Can you work these out from the model? Positions are in its coordinate system, mm. Round coordinates to 2 decimals unless told otherwise and drop trailing zeros. Loops run counter-clockwise (first coordinate to the right, second up) from the corner with the lowest first, then second, coordinate; pieces in that order, holes last. Notation, with made-up numbers: M -29,-1.75 L 4,-1.75 A28 ccw 4,28.25 Z; hole C 19.25,46.5 d1. An arc over 180 degrees is marked long. Use a Markdown table: item, result. Add a question column.
```python
from build123d import *

# Parameters (mm, degrees)
SKETCH1_W                  = 7
SKETCH1_H                  = 12
BOSS_EXTRUDE1_DEPTH        = 1.25
F_3_5_3_5_DIAMETER_HOLE1_D = 3.5
CHAMFER1_SIZE              = 1


with BuildPart() as part:
    # Sketch1 → Boss-Extrude1 (new, symmetric)
    with BuildSketch(Plane.XY):
        Rectangle(SKETCH1_W, SKETCH1_H)
    extrude(amount=BOSS_EXTRUDE1_DEPTH, both=True)

    # Ø3.5 (3.5) Diameter Hole1 (through all)
    with Locations(Plane.XY.offset(1.25)):
        with Locations((0, -3)):
            Hole(F_3_5_3_5_DIAMETER_HOLE1_D / 2)

    # Chamfer1
    chamfer1_edges = [part.edges().sort_by_distance(p)[0] for p in [
        (3.5, -6, 0),
        (-3.5, -6, 0),
        (-3.5, 6, 0),
        (3.5, 6, 0),
    ]]
    chamfer(chamfer1_edges, length=CHAMFER1_SIZE)


solid = part.part
```
(1) Suppose I cut it at B-B on x = 0. List the corners of the cut face in (y, z) for me, and give its area (4 significant figures).
(2) If I drill on probe 1 along Y at (x, z) = (0, 0.55); probe 2 along X at (y, z) = (-4.5, 0.2); probe 3 along X at (y, z) = (-3.5, -0.4), over which ranges is the centre line in solid material (lowest first)? Write a range as [from, to].
(3) I'm going to push a flat-ended pin straight in: pin 1 (4 mm diameter, centred on x = 0, y = -3, fed in from +Z). Where does the tip first touch, or does it pass through?
(4) Suppose I cut it at A-A on y = -3. List the corners of the cut face in (x, z) for me, and give its area (3 significant figures).
(5) Suppose I cut it at C-C on z = 0.95. List the corners of the cut face in (x, y) for me, and give its area (3 significant figures).
(6) Suppose I cut it at D-D on x = -3. List the corners of the cut face in (y, z) for me, and give its area (3 significant figures).
(7) Thinking about a two-plate mould opening in X: for faces 1 (the face through (0, 0, -1.25)), 2 (the face through (0.38, -4.71, -0.02)), 3 (the face through (-3, 5.5, 0)), 4 (the face through (3, 5.5, 0)), which applies, released by +X, released by -X, zero draft, split by the parting line, or undercut?
Results below:
| question | item | result |
|---|---|---|
| 1 | outline | M -6,-1.25 L -4.75,-1.25 L -4.75,1.25 L -6,1.25 Z; M -1.25,-1.25 L 6,-1.25 L 6,1.25 L -1.25,1.25 Z |
| 1 | area | 21.25 mm² |
| 2 | probe 1 | y = [-6, -4.75], [-1.25, 6] |
| 2 | probe 2 | x = [-3.5, -0.9], [0.9, 3.5] |
| 2 | probe 3 | x = [-3.5, -1.68], [1.68, 3.5] |
| 3 | pin 1 | stops at z = 1.25 |
| 4 | outline | M -3.5,-1.25 L -1.75,-1.25 L -1.75,1.25 L -3.5,1.25 Z; M 1.75,-1.25 L 3.5,-1.25 L 3.5,1.25 L 1.75,1.25 Z |
| 4 | area | 8.75 mm² |
| 5 | outline | M -3.5,-5 L -2.5,-6 L 2.5,-6 L 3.5,-5 L 3.5,5 L 2.5,6 L -2.5,6 L -3.5,5 Z; hole C 0,-3 d3.5 |
| 5 | area | 72.4 mm² |
| 6 | outline | M -5.5,-1.25 L 5.5,-1.25 L 5.5,1.25 L -5.5,1.25 Z |
| 6 | area | 27.5 mm² |
| 7 | face 1 | zero draft |
| 7 | face 2 | undercut |
| 7 | face 3 | released by -X |
| 7 | face 4 | released by +X |
